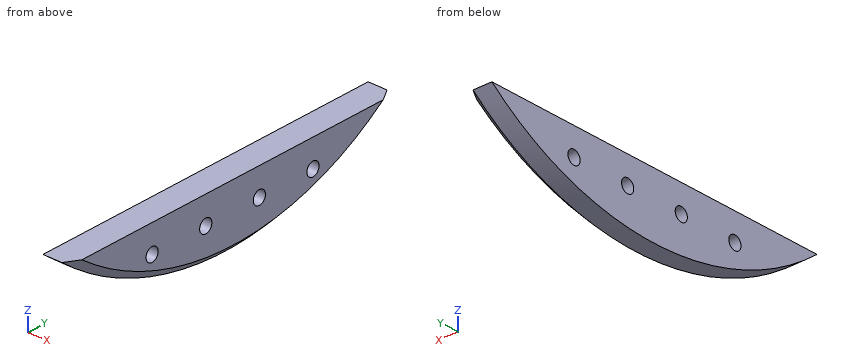
```python
from build123d import *

# Parameters (mm, degrees)
BOSS_EXTRUDE1_DEPTH = 25
SKETCH2_R           = 12.5
CUT_EXTRUDE1_DEPTH  = 81
CHAMFER2_SIZE       = 15


with BuildPart() as part:
    # Sketch1 → Boss-Extrude1 (new, symmetric)
    with BuildSketch(Plane(origin=(0, 0, 0), x_dir=(0, 0, -1), z_dir=(1, 0, 0))):
        with BuildLine():
            Line((412, 333.400659867), (412, -333.400659867))
            ThreePointArc((412, -333.400659867), (530, 0), (412, 333.400659867))
        make_face()
    extrude(amount=BOSS_EXTRUDE1_DEPTH, both=True)

    # Sketch2 → Cut-Extrude1 (cut)
    with BuildSketch(Plane(origin=(25, 0, 0), x_dir=(0, 0, -1), z_dir=(1, 0, 0))):
        with Locations((462, 55)):
            Circle(SKETCH2_R)
        with Locations((462, -55)):
            Circle(SKETCH2_R)
        with Locations((462, 165)):
            Circle(SKETCH2_R)
        with Locations((462, -165)):
            Circle(SKETCH2_R)
    extrude(amount=-CUT_EXTRUDE1_DEPTH, mode=Mode.SUBTRACT)

    # Chamfer2
    chamfer2_edges = [part.edges().sort_by_distance(p)[0] for p in [
        (25, 0, -530),
    ]]
    chamfer(chamfer2_edges, length=CHAMFER2_SIZE)


solid = part.part
```
Could you check a few things on this model? Use its own coordinates, in mm. Round coordinates to 2 decimals unless told otherwise and drop trailing zeros. Write each loop counter-clockwise with the first axis right and the second up, starting at its lowest first coordinate (ties: lowest second). Pieces come first, ordered by that corner, then holes.
(1) Suppose I cut it at B-B on z = -458. State how many separate pieces and enclosed holes the cut face has, and give its area (3 significant figures).
Findings below:
separate pieces: 5
enclosed holes: 0
area: 21,500 mm2
(2) For pin 1 (12 mm diameter, centred on x = 18, z = -447, fed in from -Y), with a flat end and sliding along its axis, tell me the tip position at first contact or that it passes through.
Findings below:
pin 1: stops at y = -284.48
(3) Suppose I cut it at A-A on x = -5. Write out the boundary of the cut face in (y, z), and give its area (3 significant figures).
Findings below:
outline: (-333.4, -412) arc R530 ccw to (333.4, -412) - close; hole circle Ø25 at (-165, -462); hole circle Ø25 at (-55, -462); hole circle Ø25 at (55, -462); hole circle Ø25 at (165, -462)
area: 51,800 mm2
(4) If I drill on probe 1 along Y at (x, z) = (-11, -462); probe 2 along Y at (x, z) = (11.5, -462); probe 3 along Z at (x, y) = (-2.5, 6.5), over which ranges is the centre line in solid material (lowest first)?
Findings below:
probe 1: y = -259.72 to -177.5, -152.5 to -67.5, -42.5 to 42.5, 67.5 to 152.5, 177.5 to 259.72
probe 2: y = -256.65 to -177.5, -152.5 to -67.5, -42.5 to 42.5, 67.5 to 152.5, 177.5 to 256.65
probe 3: z = -529.96 to -412
